Design review of the part built by this model. Coordinates are the model's own, in mm. Face numbers are marked on the shaded views. A direction names the side the tool comes from. Coordinates: 2 decimals unless noted, no trailing zeros. Write each loop counter-clockwise with the first axis right and the second up, starting at its lowest first coordinate (ties: lowest second). Pieces come first, ordered by that corner, then holes.
Q1. Take a section at D-D, the plane x = 12.5. Write out the cut boundary in (y, z).
Q2. For the marked faces 1, 2 and 3, list the 3-axis set-ups (+Z, -Z, +X, -X, +Y, -Y) from which the entire face can be reached by the end or side of a thin tool; tool diameter is ignored.
Q3. For pin 1 Ø16 at (x, y) = (-1.5, -4) entering from -Z; pin 2 Ø20.5 at (x, y) = (12.5, -9) entering from -Z; pin 3 Ø8 at (x, z) = (19, 1) entering from -Y; pin 4 Ø3 at (x, z) = (-18, 12.5) entering from -Y, all flat-tipped, find the tip position at first contact; note any pin that passes through.
Q4. The part is to be moulded in two halves that separate along Y. For the marked faces 4, 5 and 6, say which applies: released by +Y, released by -Y, zero draft, split by the parting line, or undercut.
Q5. Take a section at A-A, the plane x = 0. Write out the cut boundary in (y, z), plus the area to 3 significant figures.
Q6. Take a section at C-C, the plane z = 6.5. Write out the cut boundary in (x, y).
Q7. For L1, parallel to Y at x = 0, z = -25; L2, parallel to Y at x = 0, z = 26; L3, parallel to Z at x = -8.5, y = -12, list the stretches that pass through material, from the lowest coordinate up.
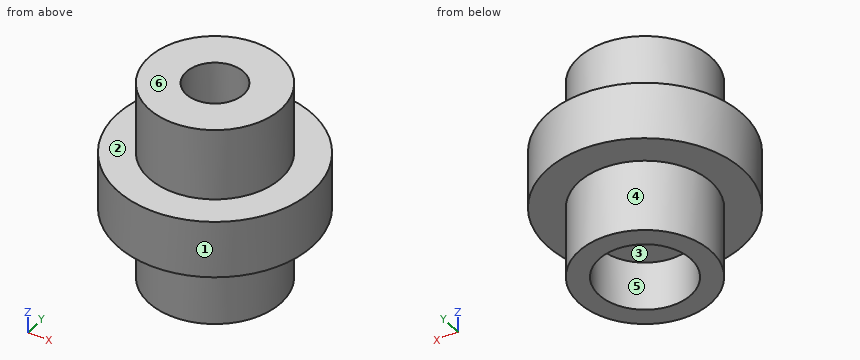
from build123d import *

# Parameters (mm, degrees)
SKETCH1_R           = 34
BOSS_EXTRUDE1_DEPTH = 10
SKETCH2_R           = 23
BOSS_EXTRUDE2_DEPTH = 25
SKETCH3_R           = 10
CUT_EXTRUDE1_DEPTH  = 17
SKETCH4_R           = 16
CUT_EXTRUDE2_DEPTH  = 17


with BuildPart() as part:
    # Sketch1 → Boss-Extrude1 (new, symmetric)
    with BuildSketch(Plane.XY):
        Circle(SKETCH1_R)
    extrude(amount=BOSS_EXTRUDE1_DEPTH, both=True)

    # Sketch2 → Boss-Extrude2 (add)
    with BuildSketch(Plane.XY.offset(10)):
        Circle(SKETCH2_R)
    boss_extrude2 = extrude(amount=BOSS_EXTRUDE2_DEPTH)

    # Mirror1: Boss-Extrude2 across plane
    add(boss_extrude2.mirror(Plane.XY))

    # Sketch3 → Cut-Extrude1 (cut)
    with BuildSketch(Plane.XY.offset(35)):
        Circle(SKETCH3_R)
    extrude(amount=-CUT_EXTRUDE1_DEPTH, mode=Mode.SUBTRACT)

    # Sketch4 → Cut-Extrude2 (cut)
    with BuildSketch(Plane(origin=(0, 0, -35), x_dir=(-1, 0, 0), z_dir=(0, 0, -1))):
        Circle(SKETCH4_R)
    extrude(amount=-CUT_EXTRUDE2_DEPTH, mode=Mode.SUBTRACT)


solid = part.part
Responses:
1. outline: (-31.62, -10) - (-19.31, -10) - (-19.31, -35) - (-9.99, -35) - (-9.99, -18) - (9.99, -18) - (9.99, -35) - (19.31, -35) - (19.31, -10) - (31.62, -10) - (31.62, 10) - (19.31, 10) - (19.31, 35) - (-19.31, 35) - (-19.31, 10) - (-31.62, 10) - close
2. face 1: +Z, -Z
2. face 2: +Z
2. face 3: -Z
3. pin 1: stops at z = -18
3. pin 2: stops at z = -35
3. pin 3: stops at y = -30.51
3. pin 4: stops at y = -16.02
4. face 4: split by the parting line
4. face 5: undercut
4. face 6: zero draft
5. outline: (-34, -10) - (-23, -10) - (-23, -35) - (-16, -35) - (-16, -18) - (16, -18) - (16, -35) - (23, -35) - (23, -10) - (34, -10) - (34, 10) - (23, 10) - (23, 35) - (10, 35) - (10, 18) - (-10, 18) - (-10, 35) - (-23, 35) - (-23, 10) - (-34, 10) - close
5. area: 2,780 mm2
6. outline: circle Ø68 at (0, 0)
7. L1: y = -23 to -16, 16 to 23
7. L2: y = -23 to -10, 10 to 23
7. L3: z = -18 to 35
